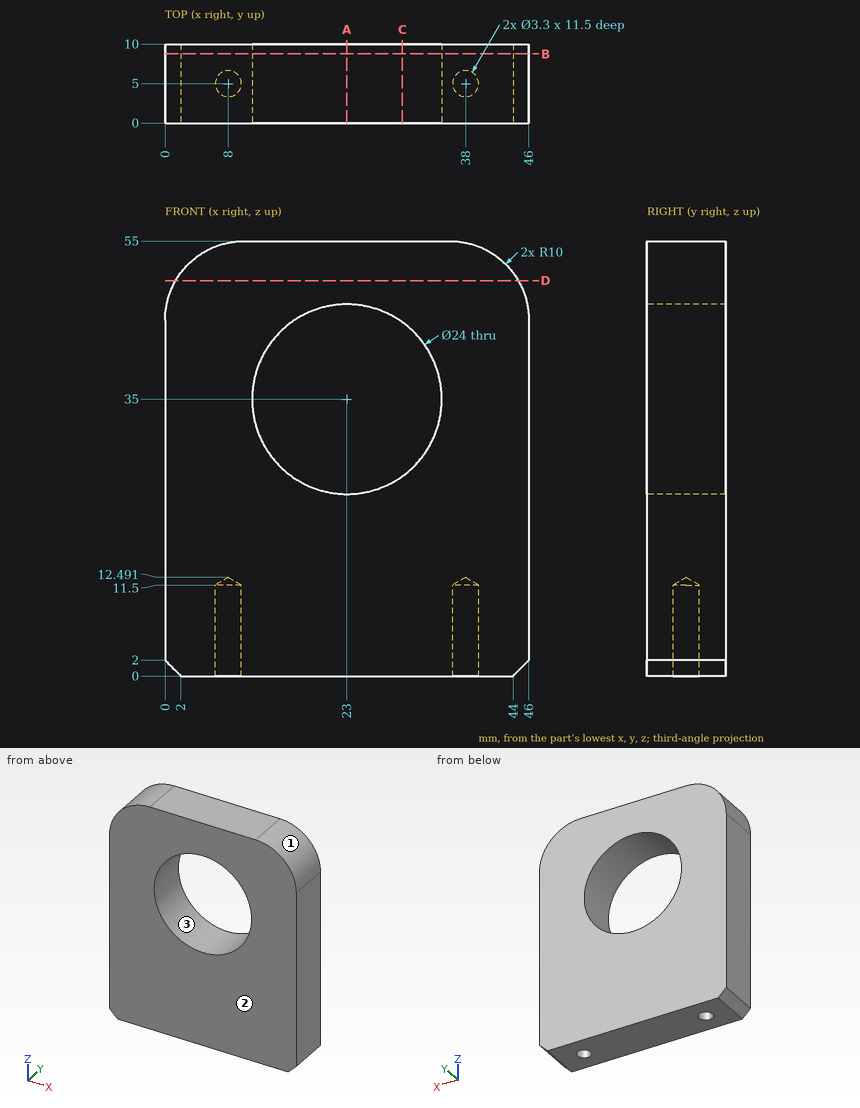
Here's the drawing with two shaded views (mm, measured from the low corner). I have some questions. Coordinates: 2 decimals unless noted, no trailing zeros. Loops run counter-clockwise (first coordinate to the right, second up) from the corner with the lowest first, then second, coordinate; pieces in that order, holes last. Notation, with made-up numbers: (5.5, 47.5) -> (31.5, 47.5) arc R28 ccw to (31.5, 68.5) -> close; hole circle Ø1 at (65.25, -39). An arc over 180 degrees is marked (long way). Answer as a JSON object with one key per item and string values.
1) If I drill on line 1 (X direction, y = 5, z = 7); line 2 (X direction, y = 4, z = 35); line 3 (Y direction, x = 38, z = 8.75), over which ranges is the centre line in solid material (lowest first)?
Results:
{"line 1": "x = 0 to 6.35, 9.65 to 36.35, 39.65 to 46", "line 2": "x = 0 to 11, 35 to 46", "line 3": "y = 0 to 3.35, 6.65 to 10"}
2) Thinking about a two-plate mould opening in Z: for the marked faces 1, 2 and 3, which applies, pulls with the +Z half, pulls with the -Z half, needs draft (parallel to the pull), parting line crosses it, or undercut?
Results:
{"face 1": "pulls with the +Z half", "face 2": "needs draft", "face 3": "undercut"}
3) Imagine slicing it at B-B (y = 8.75). Please give me the cut outline in (x, z).
Results:
{"outline": "(0, 2) -> (2, 0) -> (44, 0) -> (46, 2) -> (46, 45) arc R10 ccw to (36, 55) -> (10, 55) arc R10 ccw to (0, 45) -> close; hole circle Ø24 at (23, 35)"}
4) Imagine slicing it at A-A (x = 23). Please give me the cut outline in (y, z).
Results:
{"outline": "(0, 0) -> (10, 0) -> (10, 23) -> (0, 23) -> close; (0, 47) -> (10, 47) -> (10, 55) -> (0, 55) -> close"}
5) Imagine slicing it at D-D (z = 50). Please give me the cut outline in (x, y), then the cut area to 3 significant figures.
Results:
{"outline": "(1.34, 0) -> (44.66, 0) -> (44.66, 10) -> (1.34, 10) -> close", "area": "433 mm^2"}
6) Imagine slicing it at C-C (x = 30). Please give me the cut outline in (y, z), then the cut area to 3 significant figures.
Results:
{"outline": "(0, 0) -> (10, 0) -> (10, 25.25) -> (0, 25.25) -> close; (0, 44.75) -> (10, 44.75) -> (10, 55) -> (0, 55) -> close", "area": "355 mm^2"}
7) For P1, Ø2, axis at x = 8, y = 5, coming from the +Z side, with a flat end and sliding along its axis, tell me the tip position at first contact or that it passes through.
Results:
{"P1": "stops at z = 54.95"}
